```python
from build123d import *

# Parameters (mm, degrees)
UPRIGHT_PROFILE_SKETCH_R    = 15
UPRIGHT_BODY_DEPTH          = 50
BASE_PLATE_SKETCH_W         = 115
BASE_PLATE_SKETCH_H         = 210
BASE_PLATE_210X115X30_DEPTH = 30
BASE_BLEND_FILLET_R20_R     = 20
SIDE_BOSS_SKETCH_W          = 8
SIDE_BOSS_SKETCH_H          = 45
SIDE_BOSS_DEPTH             = 80
UPRIGHT_PROFILE_CUT_DEPTH   = 80


with BuildPart() as part:
    # Upright Profile Sketch → Upright Body (new, symmetric)
    with BuildSketch(Plane.XY):
        with BuildLine():
            Line((-40, -107.819293264), (-40, 107.819293264))
            ThreePointArc((-40, 107.819293264), (0, 115), (40, 107.819293264))
            Line((40, 107.819293264), (40, -107.819293264))
            ThreePointArc((40, -107.819293264), (35.036523196, -109.532835453), (30, -111.018016556))
            Line((30, -111.018016556), (30, -165))
            Line((30, -165), (-30, -165))
            Line((-30, -165), (-30, -111.018016556))
            ThreePointArc((-30, -111.018016556), (-35.036523196, -109.532835453), (-40, -107.819293264))
        make_face()
        with Locations((0, 75)):
            Circle(UPRIGHT_PROFILE_SKETCH_R, mode=Mode.SUBTRACT)
        with Locations(Location((0, -75, 0), (0, 0, 180))):
            Circle(UPRIGHT_PROFILE_SKETCH_R, mode=Mode.SUBTRACT)
    extrude(amount=UPRIGHT_BODY_DEPTH, both=True)

    # Base Plate Sketch → Base Plate 210x115x30 (add)
    with BuildSketch(Plane.XZ.offset(165)):
        Rectangle(BASE_PLATE_SKETCH_W, BASE_PLATE_SKETCH_H)
    extrude(amount=BASE_PLATE_210X115X30_DEPTH)

    # Base Blend Fillet R20
    base_blend_fillet_r20_edges = [part.edges().sort_by_distance(p)[0] for p in [
        (30, -165, 0),
        (-30, -165, 0),
        (0, -165, 50),
        (0, -165, -50),
    ]]
    fillet(base_blend_fillet_r20_edges, radius=BASE_BLEND_FILLET_R20_R)

    # Side Boss Sketch → Side Boss (add)
    with BuildSketch(Plane(origin=(40, 0, 0), x_dir=(0, 0, -1), z_dir=(1, 0, 0))):
        with Locations((54, 0)):
            Rectangle(SIDE_BOSS_SKETCH_W, SIDE_BOSS_SKETCH_H)
    extrude(amount=-SIDE_BOSS_DEPTH)

    # Upright Cut Sketch → Upright Profile Cut (cut)
    with BuildSketch(Plane(origin=(40, 0, 0), x_dir=(0, 0, -1), z_dir=(1, 0, 0))):
        with BuildLine():
            Line((10, 40), (-50, 40))
            Line((-50, 40), (-50, -40))
            Line((-50, -40), (10, -40))
            ThreePointArc((10, -40), (50, 0), (10, 40))
        make_face()
    extrude(amount=-UPRIGHT_PROFILE_CUT_DEPTH, mode=Mode.SUBTRACT)


solid = part.part
```
The model under review builds one solid part; all positions refer to its coordinate system, in mm. A direction names the side the tool comes from. Coordinates: 2 decimals unless noted, no trailing zeros. Write each loop counter-clockwise with the first axis right and the second up, starting at its lowest first coordinate (ties: lowest second). Pieces come first, ordered by that corner, then holes.
1) We need section D-D on y = -18. State the section outline as (x, z) points, then the cut area to 3 significant figures.
2) Machinability: for faces 5 (the face through (-30, -128, 1)), 6 (the face through (1, 40, 20)), 7 (the face through (1, 22.5, -54)), 8 (the face through (35.11, -109.51, 0.7)), 9 (the face through (1, -22.5, -54)), which of the approach directions +Z, -Z, +X, -X, +Y, -Y give a long, thin tool a straight path to every point of the face, cutting with its end or side? Answer none if there is none.
3) The part is to be moulded in two halves that separate along Y. For faces 1 (the face through (30, -128, 1)), 2 (the face through (-0.6, 115, 0.7)), 3 (the face through (-1, -180, -105)), 4 (the face through (-36.014, -159.297, 0.98)), say which applies: pulls with the +Y half, pulls with the -Y half, needs draft (parallel to the pull), parting line crosses it, or undercut.
4) Clearance check with flat-ended pins moving along their axes: pin 1 Ø8 at (x, z) = (-42.5, -27.5) entering from +Y; pin 2 Ø5 at (x, y) = (24.5, -73) entering from +Z; pin 3 Ø3 at (y, z) = (83.5, 34) entering from +X. State where each tip first meets the part, or that it passes through.
5) We need section C-C on y = 75. State the section outline as (x, z) points, then the cut area to 3 significant figures.
6) To check wall thickness, follow probe 1 along Y at (x, z) = (0, 0.5); probe 2 along Y at (x, z) = (-12.5, 30); probe 3 along Y at (x, z) = (41.5, -73). State the ranges of each line that lie inside material, in increasing order.
7) We need section B-B on x = 0. State the section outline as (y, z) points.
8) We need section A-A on z = 19. State the section outline as (x, y) points.
Answer list:
1. outline: (-40, -58) - (40, -58) - (40, -45.72) - (-40, -45.72) - close
1. area: 982 mm2
2. face 5: +Z, -Z, -X
2. face 6: +Z, +X, -X
2. face 7: -Z, +X, -X, +Y
2. face 8: +Z, -Z, +X
2. face 9: -Z, +X, -X
3. face 1: undercut
3. face 2: pulls with the +Y half
3. face 3: needs draft
3. face 4: undercut
4. pin 1: stops at y = 108.36
4. pin 2: stops at z = 50
4. pin 3: stops at x = 40
5. outline: (-40, -50) - (-15, -50) - (-15, 50) - (-40, 50) - close; (15, -50) - (40, -50) - (40, 50) - (15, 50) - close
5. area: 5,000 mm2
6. probe 1: y = -195 to -90, -60 to -40, 40 to 60, 90 to 115
6. probe 2: y = -195 to -83.29, -66.71 to -40, 40 to 66.71, 83.29 to 114.32
6. probe 3: y = -195 to -165
7. outline: (-195, -105) - (-165, -105) - (-165, -70) arc R20 cw to (-145, -50) - (-90, -50) - (-90, 50) - (-145, 50) arc R20 cw to (-165, 70) - (-165, 105) - (-195, 105) - close; (-60, -50) - (-22.5, -50) - (-22.5, -58) - (22.5, -58) - (22.5, -50) - (60, -50) - (60, 50) - (40, 50) - (40, -10) arc R40 cw to (-40, -10) - (-40, 50) - (-60, 50) - close; (90, -50) - (115, -50) - (115, 50) - (90, 50) - close
8. outline: (-57.5, -195) - (57.5, -195) - (57.5, -165) - (50, -165) arc R20 cw to (30, -145) - (30, -111.02) arc R115 ccw to (40, -107.82) - (40, -40) - (-40, -40) - (-40, -107.82) arc R115 ccw to (-30, -111.02) - (-30, -145) arc R20 cw to (-50, -165) - (-57.5, -165) - close; (-40, 40) - (40, 40) - (40, 107.82) arc R115 ccw to (-40, 107.82) - close; hole circle Ø30 at (0, -75); hole circle Ø30 at (0, 75)
